Input: part model. Units: mm. Frame: model coordinates. Face numbers are marked on the shaded views. A direction names the side the tool comes from. Coordinates: 2 decimals unless noted, no trailing zeros. Loops run counter-clockwise (first coordinate to the right, second up) from the corner with the lowest first, then second, coordinate; pieces in that order, holes last.
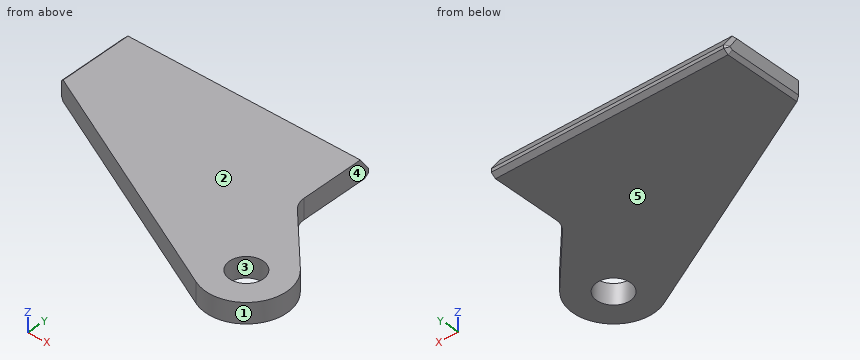
```python
from build123d import *

# Parameters (mm, degrees)
SKETCH_1_R          = 25
EXTRUDE_1_DEPTH     = 30
CUT_EXTRUDE_2_DEPTH = 516.654923374
CUT_EXTRUDE_3_DEPTH = 516.654923374
CHAMFER_1_SIZE      = 5
FILLET_2_R          = 30


with BuildPart() as part:
    # 草图1 → 凸台-拉伸1 (new body)
    with BuildSketch(Plane.XY):
        with BuildLine():
            Line((-40, 250), (-390, 250))
            Line((-390, 250), (-390, 130))
            Line((-390, 130), (-27.078184069, -53.542244514))
            ThreePointArc((-27.078184069, -53.542244514), (48.059978328, -35.919889798), (43.681693947, 41.132828907))
            Line((43.681693947, 41.132828907), (-40, 130))
            Line((-40, 130), (-40, 250))
        make_face()
        Circle(SKETCH_1_R, mode=Mode.SUBTRACT)
    extrude(amount=EXTRUDE_1_DEPTH)

    # 草图2 → 切除-拉伸2 (cut, through all)
    with BuildSketch(Plane(origin=(60, 0, 0), x_dir=(0, 0, -1), z_dir=(1, 0, 0))):
        Polygon((-10, 250), (-30, 235.995849236), (-30, 250), align=None)
    extrude(amount=-CUT_EXTRUDE_2_DEPTH, mode=Mode.SUBTRACT)

    # 草图3 → 切除-拉伸3 (cut, through all)
    with BuildSketch(Plane(origin=(60, 0, 0), x_dir=(0, 0, -1), z_dir=(1, 0, 0))):
        Polygon((-5, 250), (0, 242.859259966), (0, 250), align=None)
    extrude(amount=-CUT_EXTRUDE_3_DEPTH, mode=Mode.SUBTRACT)

    # 倒角1
    chamfer_1_edges = [part.edges().sort_by_distance(p)[0] for p in [
        (-390, 182.997924618, 30),
        (-390, 250, 7.5),
        (-390, 242.997924618, 20),
        (-390, 186.429629983, 0),
        (-390, 246.429629983, 2.5),
    ]]
    chamfer(chamfer_1_edges, length=CHAMFER_1_SIZE)

    # 圆角2
    fillet_2_edges = [part.edges().sort_by_distance(p)[0] for p in [
        (-40, 130, 15),
    ]]
    fillet(fillet_2_edges, radius=FILLET_2_R)


solid = part.part
```
Item 1: Mould query, pull axis Y, two halves, no side actions, for the marked faces 1, 2 and 3. Classes: +Y half, -Y half, draft (parallel to the pull), parting line (faces both ways), or undercut.
Result:
face 1: parting line
face 2: draft
face 3: undercut
Item 2: Line query: L1, parallel to Y at x = 0, z = 16; L2, parallel to X at y = 156, z = 23; L3, parallel to Y at x = -102.5, z = 11.5. Output: solid intervals per line, ascending.
Result:
L1: y = -60 to -25, 25 to 87.52
L2: x = -390 to -40
L3: y = -15.4 to 248.95
Item 3: Section query A-A (y = 0). Output: boundary loops of the cut face in (x, z).
Result:
outline: (-132.95, 0) - (-25, 0) - (-25, 30) - (-132.95, 30) - close; (25, 0) - (60, 0) - (60, 30) - (25, 30) - close
Item 4: Section query C-C (y = 223.5). Output: boundary loops of the cut face in (x, z), then the cut area to 3 significant figures.
Result:
outline: (-390, 5) - (-385, 0) - (-40, 0) - (-40, 30) - (-385, 30) - (-390, 25) - close
area: 10,500 mm2
Item 5: Contact query for flat-ended pins moving along their axis: P1, Ø1, axis at x = -126, z = 13.5, coming from the -Y side; P2, Ø9, axis at y = 205.5, z = 13, coming from the +X side; P3, Ø10, axis at x = -74, z = 22, coming from the -Y side. Output: stop coordinate, or through.
Result:
P1: stops at y = -3.77
P2: stops at x = -40
P3: stops at y = -32.34
Item 6: Section query B-B (x = 8). Output: boundary loops of the cut face in (y, z).
Result:
outline: (-59.46, 0) - (-23.69, 0) - (-23.69, 30) - (-59.46, 30) - close; (23.69, 0) - (79.03, 0) - (79.03, 30) - (23.69, 30) - close
Item 7: Reachability of the marked faces 4 and 5 from +Z, -Z, +X, -X, +Y, -Y: full face, straight path, thin tool, end or side. Return the list, or none.
Result:
face 4: +Z, -Z, +X, +Y
face 5: -Z, +X, -X, +Y, -Y
Item 8: Section query D-D (x = -133). Output: boundary loops of the cut face in (y, z).
Result:
outline: (0.03, 0) - (242.86, 0) - (250, 5) - (250, 10) - (236, 30) - (0.03, 30) - close
